Source: CAD feature listing. Evaluate the final solid. Frame: model axes, mm. Give positions to 0.01 mm unless a question says otherwise; leave off trailing zeros. Loops run counter-clockwise (first coordinate to the right, second up) from the corner with the lowest first, then second, coordinate; pieces in that order, holes last. Notation, with made-up numbers: M 24,78 L 51,78 A14 cw 51,89 Z; hole C -23,87 d7. An arc over 180 degrees is marked long. Answer in a Markdown table with one row per item.
```python
from build123d import *

# Parameters (mm, degrees)
SKETCH1_R               = 15
BOSS_EXTRUDE1_DEPTH     = 130
SKETCH2_R               = 20
BOSS_EXTRUDE2_DEPTH     = 10
CUT_EXTRUDE1_DEPTH      = 143.828568571
CUT_EXTRUDE1_DEPTH_BACK = 143.828568571
SKETCH3_R               = 4
CHAMFER1_SIZE           = 2
FILLET1_R               = 1
FILLET2_R               = 1


with BuildPart() as part:
    # Sketch1 → Boss-Extrude1 (new body)
    with BuildSketch(Plane.XY):
        Circle(SKETCH1_R)
    extrude(amount=BOSS_EXTRUDE1_DEPTH)

    # Sketch2 → Boss-Extrude2 (add)
    with BuildSketch(Plane.XY.offset(130)):
        Circle(SKETCH2_R)
    extrude(amount=BOSS_EXTRUDE2_DEPTH)

    # Sketch3 → Cut-Extrude1 (cut, two sides: drawn at the far end of the back side and taken through both)
    with BuildSketch(Plane(origin=(0, 0, 0), x_dir=(1, 0, 0), z_dir=(0, 1, 0)).offset(-CUT_EXTRUDE1_DEPTH_BACK)):
        with Locations(Location((0, -10, 0), (0, 0, 270))):
            Circle(SKETCH3_R)
    extrude(amount=CUT_EXTRUDE1_DEPTH + CUT_EXTRUDE1_DEPTH_BACK, mode=Mode.SUBTRACT)

    # Chamfer1
    chamfer1_edges = [part.edges().sort_by_distance(p)[0] for p in [
        (-15, 0, 0),
    ]]
    chamfer(chamfer1_edges, length=CHAMFER1_SIZE)

    # Fillet1
    fillet1_edges = [part.edges().sort_by_distance(p)[0] for p in [
        (-15, 0, 130),
    ]]
    fillet(fillet1_edges, radius=FILLET1_R)

    # Fillet2
    fillet2_edges = [part.edges().sort_by_distance(p)[0] for p in [
        (-20, 0, 130),
        (-20, 0, 140),
    ]]
    fillet(fillet2_edges, radius=FILLET2_R)


solid = part.part
```
1) Section C-C, the plane z = 10. Return loops of the section in (x, y), then the cut area to 3 significant figures.
Reply:
| item | result |
|---|---|
| outline | M -4,-14.46 L -4,14.46 A15 ccw Z; M 4,-14.46 A15 ccw 4,14.46 Z |
| area | 470 mm² |
2) Section B-B, the plane y = 0. Return loops of the section in (x, z).
Reply:
| item | result |
|---|---|
| outline | M -20,131 A1 ccw -19,130 L -16,130 A1 cw -15,129 L -15,2 L -13,0 L 13,0 L 15,2 L 15,129 A1 cw 16,130 L 19,130 A1 ccw 20,131 L 20,139 A1 ccw 19,140 L -19,140 A1 ccw -20,139 Z; hole C 0,10 d8 |
3) Material intervals for L1, parallel to Z at x = 0, y = -3; L2, parallel to Z at x = 2.5, y = -9.5; L3, parallel to X at y = -3, z = 10, sorted ascending.
Reply:
| item | result |
|---|---|
| L1 | z = 0 to 6, 14 to 140 |
| L2 | z = 0 to 6.88, 13.12 to 140 |
| L3 | x = -14.7 to -4, 4 to 14.7 |
4) Section D-D, the plane z = 110. Return loops of the section in (x, y).
Reply:
| item | result |
|---|---|
| outline | C 0,0 d30 |
5) Pin query (flat end, axial travel): pin 1 Ø4 at (y, z) = (5, 29) entering from +X; pin 2 Ø6 at (x, z) = (-9, 16) entering from -Y; pin 3 Ø4 at (y, z) = (-5.5, 20.5) entering from +X. Return the tip coordinate at first contact, or that it passes through.
Reply:
| item | result |
|---|---|
| pin 1 | stops at x = 14.7 |
| pin 2 | stops at y = -13.75 |
| pin 3 | stops at x = 14.59 |
6) Section A-A, the plane x = 0. Return loops of the section in (y, z), then the cut area to 3 significant figures.
Reply:
| item | result |
|---|---|
| outline | M -20,131 A1 ccw -19,130 L -16,130 A1 cw -15,129 L -15,14 L 15,14 L 15,129 A1 cw 16,130 L 19,130 A1 ccw 20,131 L 20,139 A1 ccw 19,140 L -19,140 A1 ccw -20,139 Z; M -15,2 L -13,0 L 13,0 L 15,2 L 15,6 L -15,6 Z |
| area | 4,060 mm² |
7) Pull-direction query (Z, two-part tool) for faces 1 (the flat face through (0, 0, 140)), 2 (the cylindrical face through (-4.336, -19.524, 134.944)), 3 (the cylindrical face through (0, 0, 6)), 4 (the flat face through (0, 0, 0)); classes: released by +Z, released by -Z, zero draft, split by the parting line, or undercut.
Reply:
| item | result |
|---|---|
| face 1 | released by +Z |
| face 2 | zero draft |
| face 3 | undercut |
| face 4 | released by -Z |
